```python
from build123d import *

# Parameters (mm, degrees)
EXTRUDE_1_DEPTH              = 50
CHAMFER_1_SIZE               = 1
HOLE_WIZARD_M3_1_D           = 3.4
HOLE_WIZARD_M3_1_CBORE_D     = 6
HOLE_WIZARD_M3_1_CBORE_DEPTH = 3.4


with BuildPart() as part:
    # 草图1 → 凸台-拉伸1 (new body)
    with BuildSketch(Plane(origin=(0, 0, 0), x_dir=(1, 0, 0), z_dir=(0, 1, 0))):
        Polygon((10, 0), (-10, 0), (-10, 5), (-6, 5), (-6, 10), (6, 10), (6, 5), (10, 5), align=None)
    extrude(amount=EXTRUDE_1_DEPTH)

    # 倒角1
    chamfer_1_edges = [part.edges().sort_by_distance(p)[0] for p in [
        (8, 0, -5),
        (10, 0, -2.5),
        (0, 0, 0),
        (-10, 0, -2.5),
        (10, 50, -2.5),
        (8, 50, -5),
        (6, 50, -7.5),
        (0, 50, -10),
        (-6, 50, -7.5),
        (-8, 50, -5),
        (-10, 50, -2.5),
        (-8, 0, -5),
        (0, 50, 0),
        (-6, 0, -7.5),
        (0, 0, -10),
        (6, 0, -7.5),
    ]]
    chamfer(chamfer_1_edges, length=CHAMFER_1_SIZE)

    # M3 六角圆柱头螺钉的柱形沉头孔1 (through all)
    with Locations(Plane.XY):
        with Locations((0, 42.5), (0, 7.5)):
            CounterBoreHole(HOLE_WIZARD_M3_1_D / 2, HOLE_WIZARD_M3_1_CBORE_D / 2, HOLE_WIZARD_M3_1_CBORE_DEPTH)


solid = part.part
```
Geometry check sheet. Reference: the model listing, model coordinates, mm. A direction names the side the tool comes from. Give positions to 0.01 mm unless a question says otherwise; leave off trailing zeros. Order: outer loops, then holes, each group sorted by start corner. A loop starts at its lowest first (then second) coordinate and runs counter-clockwise, first axis right, second up. Notation, with made-up numbers: (-30, 83.25) - (20, 83.25) arc R22 ccw to (20, 114.25) - close; hole circle Ø6 at (-26, 69). An arc over 180 degrees is marked (long way). Answer in a Markdown table with one row per item. Add a question column.
Q1. Cross-section at D-D, the plane y = 16. Enter the section's corners in (x, z), then the cut area to 3 significant figures.
Q2. Cross-section at C-C, the plane x = 0. Enter the section's corners in (y, z).
Q3. Cross-section at A-A, the plane z = -7. Enter the section's corners in (x, y).
Q4. Material ranges on probe 1 along Y at (x, z) = (0, -7.25); probe 2 along Y at (x, z) = (0, -1.1); probe 3 along Z at (x, y) = (7.75, 43), recorded low to high. Write a range as from..to.
Q5. Tool access check on faces 5 (the flat face through (-7.5, 49.5, -4.5)), 6 (the flat face through (8, 25, -5)), 7 (the flat face through (5.5, 49.5, -7)). Record the directions out of +Z, -Z, +X, -X, +Y, -Y that give a thin tool (end or side, any length) a straight path to the whole face; none if there is none.
Q6. Mould release check, pull along Y, two halves, no side actions. Record for faces 1 (the cylindrical face through (-3, 7.6, -1.7)), 2 (the flat face through (7.5, 0.5, -4.5)), 3 (the flat face through (-8, 25, -5)), 4 (the flat face through (-9.5, 49.5, -2.5)): pulls with the +Y half, pulls with the -Y half, needs draft (parallel to the pull), parting line crosses it, or undercut.
Q7. Gauge pin test, flat ends, axial feed: pin 1 (5.5 mm diameter, centred on y = 33, z = -8, fed in from -X); pin 2 (2 mm diameter, centred on x = -9, y = 15, fed in from -Z); pin 3 (1.8 mm diameter, centred on x = 1, y = 7, fed in from +Z). Record the tip position at first contact, or that the pin passes through.
Q8. Cross-section at B-B, the plane y = 42.5. Enter the section's corners in (x, z).
Check values:
| question | item | result |
|---|---|---|
| 1 | outline | (-10, -5) - (-6, -5) - (-6, -10) - (6, -10) - (6, -5) - (10, -5) - (10, 0) - (-10, 0) - close |
| 1 | area | 160 mm^2 |
| 2 | outline | (0, -9) - (1, -10) - (5.8, -10) - (5.8, -3.4) - (4.5, -3.4) - (4.5, 0) - (1, 0) - (0, -1) - close; (9.2, -10) - (40.8, -10) - (40.8, -3.4) - (39.5, -3.4) - (39.5, 0) - (10.5, 0) - (10.5, -3.4) - (9.2, -3.4) - close; (44.2, -10) - (49, -10) - (50, -9) - (50, -1) - (49, 0) - (45.5, 0) - (45.5, -3.4) - (44.2, -3.4) - close |
| 3 | outline | (-6, 1) - (-5, 0) - (5, 0) - (6, 1) - (6, 49) - (5, 50) - (-5, 50) - (-6, 49) - close; hole circle Ø3.4 at (0, 7.5); hole circle Ø3.4 at (0, 42.5) |
| 4 | probe 1 | y = 0..5.8, 9.2..40.8, 44.2..50 |
| 4 | probe 2 | y = 0..4.5, 10.5..39.5, 45.5..50 |
| 4 | probe 3 | z = -5..0 |
| 5 | face 5 | -Z, -X, +Y |
| 5 | face 6 | -Z, +X, +Y, -Y |
| 5 | face 7 | -Z, +X, +Y |
| 6 | face 1 | undercut |
| 6 | face 2 | pulls with the -Y half |
| 6 | face 3 | needs draft |
| 6 | face 4 | pulls with the +Y half |
| 7 | pin 1 | stops at x = -6 |
| 7 | pin 2 | stops at z = -5 |
| 7 | pin 3 | stops at z = -3.4 |
| 8 | outline | (-10, -5) - (-6, -5) - (-6, -10) - (-1.7, -10) - (-1.7, -3.4) - (-3, -3.4) - (-3, 0) - (-10, 0) - close; (1.7, -10) - (6, -10) - (6, -5) - (10, -5) - (10, 0) - (3, 0) - (3, -3.4) - (1.7, -3.4) - close |
